Read the model definition and answer for the solid it produces. Units are mm, in the model's axes. A direction names the side the tool comes from. Round coordinates to 2 decimals unless told otherwise and drop trailing zeros. Write each loop counter-clockwise with the first axis right and the second up, starting at its lowest first coordinate (ties: lowest second). Pieces come first, ordered by that corner, then holes. Notation, with made-up numbers: (32.5, 30.25) - (57.5, 30.25) arc R17 ccw to (57.5, 54.25) - close; hole circle Ø9 at (74, 7). An arc over 180 degrees is marked (long way). Use one line per item in the form item = value. Start each with the question number.
1) The part is cut by section A-A, the plane y = 1.5. Give the vertices of the cut face in (x, z), plus the area to 3 significant figures.
2) Consider line 1 along Y through (x, z) = (-2, 6.75); line 2 along Z through (x, y) = (4.5, 0.5). Determine where each line is inside the solid, lowest interval first. Write a range as from..to.
3) For a pull along X with two mould halves and no side action, classify faces 4 (the face through (0, 3, 15)), 5 (the face through (5, 0, 7)), 6 (the face through (0, -4, 1.5)) as released by +X, released by -X, zero draft, split by the parting line, or undercut.
4) For faces 1 (the face through (0, 2.5, 1)), 2 (the face through (2.5, 0, 4)), 3 (the face through (0, -4, 6.5)), determine the directions among +Z, -Z, +X, -X, +Y, -Y from which every point of the face is accessible in a straight line to the end or side of a thin tool.
5) The part is cut by section D-D, the plane z = 1.25. Give the vertices of the cut face in (x, y), plus the area to 3 significant figures.
6) The part is cut by section B-B, the plane z = 4.5. Give the vertices of the cut face in (x, y).
7) The part is cut by section C-C, the plane x = 2. Give the vertices of the cut face in (y, z).
from build123d import *

# Parameters (mm, degrees)
SKETCH1_W           = 10
SKETCH1_H           = 10
SKETCH1_W_2         = 5
SKETCH1_H_2         = 5
BOSS_EXTRUDE1_DEPTH = 15
SKETCH2_W           = 5
SKETCH2_H           = 5
CUT_EXTRUDE1_DEPTH  = 19.708286934
SKETCH3_W           = 5
SKETCH3_H           = 5
CUT_EXTRUDE2_DEPTH  = 19.708286934


with BuildPart() as part:
    # Sketch1 → Boss-Extrude1 (new body)
    with BuildSketch(Plane.XY):
        Rectangle(SKETCH1_W, SKETCH1_H)
        Rectangle(SKETCH1_W_2, SKETCH1_H_2, mode=Mode.SUBTRACT)
    extrude(amount=BOSS_EXTRUDE1_DEPTH)

    # Sketch2 → Cut-Extrude1 (cut, through all)
    with BuildSketch(Plane(origin=(0, 5, 0), x_dir=(1, 0, 0), z_dir=(0, 1, 0))):
        with Locations((0, -4)):
            Rectangle(SKETCH2_W, SKETCH2_H)
    extrude(amount=-CUT_EXTRUDE1_DEPTH, mode=Mode.SUBTRACT)

    # Sketch3 → Cut-Extrude2 (cut, through all)
    with BuildSketch(Plane(origin=(5, 0, 0), x_dir=(0, 0, -1), z_dir=(1, 0, 0))):
        with Locations((-11, 0)):
            Rectangle(SKETCH3_W, SKETCH3_H)
    extrude(amount=-CUT_EXTRUDE2_DEPTH, mode=Mode.SUBTRACT)


solid = part.part
Geometry results:
q1.outline = (-5, 0) - (-2.5, 0) - (-2.5, 8.5) - (-5, 8.5) - close; (-5, 13.5) - (-2.5, 13.5) - (-2.5, 15) - (-5, 15) - close; (2.5, 0) - (5, 0) - (5, 8.5) - (2.5, 8.5) - close; (2.5, 13.5) - (5, 13.5) - (5, 15) - (2.5, 15) - close
q1.area = 50.0 mm2
q2.line_1 = -5..-2.5, 2.5..5
q2.line_2 = 0..8.5, 13.5..15
q3.face_4 = zero draft
q3.face_5 = released by +X
q3.face_6 = undercut
q4.face_1 = +Z, -Z
q4.face_2 = none
q4.face_3 = +Y, -Y
q5.outline = (-5, -5) - (5, -5) - (5, 5) - (-5, 5) - close; hole (-2.5, -2.5) - (2.5, -2.5) - (2.5, 2.5) - (-2.5, 2.5) - close
q5.area = 75.0 mm2
q6.outline = (-5, -5) - (-2.5, -5) - (-2.5, 5) - (-5, 5) - close; (2.5, -5) - (5, -5) - (5, 5) - (2.5, 5) - close
q7.outline = (-5, 0) - (-2.5, 0) - (-2.5, 1.5) - (-5, 1.5) - close; (-5, 6.5) - (-2.5, 6.5) - (-2.5, 15) - (-5, 15) - close; (2.5, 0) - (5, 0) - (5, 1.5) - (2.5, 1.5) - close; (2.5, 6.5) - (5, 6.5) - (5, 15) - (2.5, 15) - close
